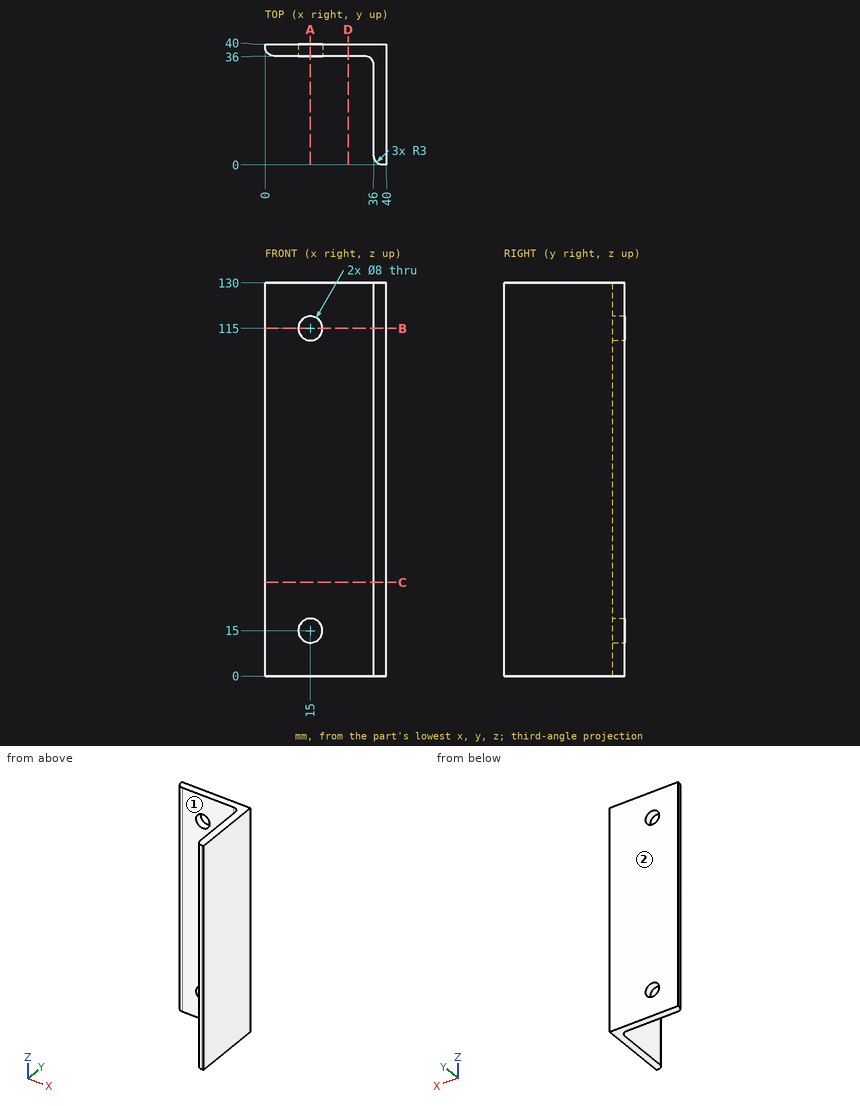
Check sheet for the drawn part. Datum: minimum x, y, z corner. Units: mm. A direction names the side the tool comes from. Coordinates: 2 decimals unless noted, no trailing zeros. Loops run counter-clockwise (first coordinate to the right, second up) from the corner with the lowest first, then second, coordinate; pieces in that order, holes last. Notation, with made-up numbers: (52, 64.25) -> (62, 64.25) arc R11 cw to (62, 72.25) -> close; hole circle Ø1 at (74, 53). An arc over 180 degrees is marked (long way). Answer as CSV lines item,"result".
1) Cross-section at D-D, the plane x = 27.5. Record the cut outline in (y, z), then the cut area to 3 significant figures.
Found:
outline,"(36, 0) -> (40, 0) -> (40, 130) -> (36, 130) -> close"
area,"520 mm2"
2) Cross-section at C-C, the plane z = 31. Record the cut outline in (x, y).
Found:
outline,"(0, 39) arc R3 ccw to (3, 36) -> (33, 36) arc R3 cw to (36, 33) -> (36, 3) arc R3 ccw to (39, 0) -> (40, 0) -> (40, 40) -> (0, 40) -> close"
3) Cross-section at A-A, the plane x = 15. Record the cut outline in (y, z).
Found:
outline,"(36, 0) -> (40, 0) -> (40, 11) -> (36, 11) -> close; (36, 19) -> (40, 19) -> (40, 111) -> (36, 111) -> close; (36, 119) -> (40, 119) -> (40, 130) -> (36, 130) -> close"
4) Thickness scan on L1, parallel to X at y = 11.5, z = 30; L2, parallel to X at y = 37.8, z = 15. Record the ranges inside material, lowest first. Write a range as from..to.
Found:
L1,"x = 36..40"
L2,"x = 0.25..11, 19..40"
5) Tool access check on the marked faces 1 and 2. Record the directions out of +Z, -Z, +X, -X, +Y, -Y that give a thin tool (end or side, any length) a straight path to the whole face; none if there is none.
Found:
face 1,"+Z, -Z, -X, -Y"
face 2,"+Z, -Z, +X, -X, +Y"
6) Cross-section at B-B, the plane z = 115. Record the cut outline in (x, y), then the cut area to 3 significant figures.
Found:
outline,"(0, 39) arc R3 ccw to (3, 36) -> (11, 36) -> (11, 40) -> (0, 40) -> close; (19, 36) -> (33, 36) arc R3 cw to (36, 33) -> (36, 3) arc R3 ccw to (39, 0) -> (40, 0) -> (40, 40) -> (19, 40) -> close"
area,"270 mm2"
7) Depth check by flat-ended pin: pin 1 (12 mm diameter, centred on x = 10, z = 69.5, fed in from -Y); pin 2 (3 mm diameter, centred on y = 8, z = 89.5, fed in from -X). Enter the tip coordinate at first touch or a pass-through.
Found:
pin 1,"stops at y = 36"
pin 2,"stops at x = 36"
